```python
from build123d import *

# Parameters (mm, degrees)
BOSS_EXTRUDE1_DEPTH = 12


with BuildPart() as part:
    # Sketch1 → Boss-Extrude1 (new body)
    with BuildSketch(Plane.XY):
        with BuildLine():
            Line((0, 10), (0, 578))
            Line((0, 578), (96, 578))
            Line((96, 578), (60.5, 0))
            Line((60.5, 0), (10, 0))
            ThreePointArc((10, 0), (2.928932188, 2.928932188), (0, 10))
        make_face()
    extrude(amount=BOSS_EXTRUDE1_DEPTH)


solid = part.part
```
Could you check a few things on this model? Use its own coordinates, in mm. Give positions to 0.01 mm unless a question says otherwise; leave off trailing zeros. Order: outer loops, then holes, each group sorted by start corner. A loop starts at its lowest first (then second) coordinate and runs counter-clockwise, first axis right, second up.
Q1. Suppose I cut it at C-C, the plane x = 78. Write out the boundary of the cut face in (y, z), and give its area (3 significant figures).
Q2. Suppose I cut it at B-B, the plane y = 323. Write out the boundary of the cut face in (x, z).
Q3. I'm going to push a flat-ended pin straight in: P1, Ø6, axis at y = 149.5, z = 5.5, coming from the +X side. Where does the tip first touch, or does it pass through?
Q4. If I drill on line 1 along X through (y, z) = (325, 8.5); line 2 along X through (y, z) = (267.5, 10.5); line 3 along Y through (x, z) = (8.5, 10.5), over which ranges is the centre line in solid material (lowest first)?
Q5. Suppose I cut it at A-A, the plane z = 3.25. Write out the boundary of the cut face in (x, y).
Solution:
1. outline: (284.93, 0) - (578, 0) - (578, 12) - (284.93, 12) - close
1. area: 3,520 mm2
2. outline: (0, 0) - (80.34, 0) - (80.34, 12) - (0, 12) - close
3. P1: stops at x = 69.87
4. line 1: x = 0 to 80.46
4. line 2: x = 0 to 76.93
4. line 3: y = 0.11 to 578
5. outline: (0, 10) arc R10 ccw to (10, 0) - (60.5, 0) - (96, 578) - (0, 578) - close
